Design review of the part built by this model. Coordinates are the model's own, in mm. A direction names the side the tool comes from. Coordinates: 2 decimals unless noted, no trailing zeros. Write each loop counter-clockwise with the first axis right and the second up, starting at its lowest first coordinate (ties: lowest second). Pieces come first, ordered by that corner, then holes. Notation, with made-up numbers: (-14, 46.5) -> (13, 46.5) arc R32 ccw to (13, 72.5) -> close; hole circle Ø2 at (37, 37). An arc over 180 degrees is marked (long way). Answer in a Markdown table with one row per item. Add a question column.
Item 1: For faces 1 (the face through (47.03, 166.91, 82.79)), 2 (the face through (-1, 2, 0)), 3 (the face through (-1, 166.3, 45)), list the 3-axis set-ups (+Z, -Z, +X, -X, +Y, -Y) from which the entire face can be reached by the end or side of a thin tool; tool diameter is ignored.
Item 2: Take a section at B-B, the plane y = -145.5. Write out the cut boundary in (x, z), and give its area (3 significant figures).
Item 3: Draft analysis for pull direction X (two halves, no side actions). For faces 4 (the face through (-1, 167.5, 44)), 5 (the face through (-80, -2, 44)), 6 (the face through (-78.8, -2, 45)), state which applies: released by +X, released by -X, zero draft, split by the parting line, or undercut.
Item 4: Clearance check with flat-ended pins moving along their axes: P1, Ø1, axis at x = -79.5, y = 105.5, coming from the -Z side; P2, Ø4, axis at x = -18, y = -50, coming from the +Z side. State where each tip first meets the part, or that it passes through.
Item 5: To check wall thickness, follow line 1 (X direction, y = -45, z = 48.5); line 2 (Y direction, x = -41.5, z = 17.5); line 3 (X direction, y = 167, z = 85). State the ranges of each line that lie inside material, in increasing order.
Item 6: Take a section at A-A, the plane z = 42. Write out the cut boundary in (x, y), and give its area (3 significant figures).
from build123d import *

# Parameters (mm, degrees)
SKETCH1_W           = 160
SKETCH1_H           = 335
BOSS_EXTRUDE1_DEPTH = 90
SHELL1_T            = -1.2
SKETCH2_R           = 3
CUT_EXTRUDE1_DEPTH  = 10
CUT_EXTRUDE2_DEPTH  = 249.508048159


with BuildPart() as part:
    # Sketch1 → Boss-Extrude1 (new body)
    with BuildSketch(Plane.XY):
        Rectangle(SKETCH1_W, SKETCH1_H)
    extrude(amount=BOSS_EXTRUDE1_DEPTH)

    # Shell1
    shell1_openings = [part.faces().sort_by_distance(p)[0] for p in [
        (0, 0, 90),
    ]]
    offset(amount=SHELL1_T, openings=shell1_openings, kind=Kind.INTERSECTION)

    # Sketch2 → Cut-Extrude1 (cut)
    with BuildSketch(Plane(origin=(0, 167.5, 0), x_dir=(1, 0, 0), z_dir=(0, 1, 0))):
        with Locations(Location((-45, -85, 0), (0, 0, 270))):
            Circle(SKETCH2_R)
        with Locations(Location((-25, -85, 0), (0, 0, 270))):
            Circle(SKETCH2_R)
        with Locations(Location((25, -85, 0), (0, 0, 270))):
            Circle(SKETCH2_R)
        with Locations(Location((45, -85, 0), (0, 0, 270))):
            Circle(SKETCH2_R)
    extrude(amount=-CUT_EXTRUDE1_DEPTH, mode=Mode.SUBTRACT)

    # Sketch3 → Cut-Extrude2 (cut, through all)
    with BuildSketch(Plane.ZY.offset(80)):
        with BuildLine():
            Line((87.8, 106.5), (87.8, 103.5))
            ThreePointArc((87.8, 103.5), (85, 100.7), (82.2, 103.5))
            Line((82.2, 103.5), (82.2, 106.5))
            ThreePointArc((82.2, 106.5), (85, 109.3), (87.8, 106.5))
        make_face()
        with BuildLine():
            Line((87.8, -106.5), (87.8, -103.5))
            ThreePointArc((87.8, -103.5), (85, -100.7), (82.2, -103.5))
            Line((82.2, -103.5), (82.2, -106.5))
            ThreePointArc((82.2, -106.5), (85, -109.3), (87.8, -106.5))
        make_face()
    extrude(amount=-CUT_EXTRUDE2_DEPTH, mode=Mode.SUBTRACT)


solid = part.part
Answers:
| question | item | result |
|---|---|---|
| 1 | face 1 | +Y |
| 1 | face 2 | -Z, +X, -X, +Y, -Y |
| 1 | face 3 | +Z |
| 2 | outline | (-80, 0) -> (80, 0) -> (80, 90) -> (78.8, 90) -> (78.8, 1.2) -> (-78.8, 1.2) -> (-78.8, 90) -> (-80, 90) -> close |
| 2 | area | 405 mm^2 |
| 3 | face 4 | zero draft |
| 3 | face 5 | released by -X |
| 3 | face 6 | undercut |
| 4 | P1 | stops at z = 0 |
| 4 | P2 | stops at z = 1.2 |
| 5 | line 1 | x = -80 to -78.8, 78.8 to 80 |
| 5 | line 2 | y = -167.5 to -166.3, 166.3 to 167.5 |
| 5 | line 3 | x = -80 to -48, -42 to -28, -22 to 22, 28 to 42, 48 to 80 |
| 6 | outline | (-80, -167.5) -> (80, -167.5) -> (80, 167.5) -> (-80, 167.5) -> close; hole (-78.8, -166.3) -> (78.8, -166.3) -> (78.8, 166.3) -> (-78.8, 166.3) -> close |
| 6 | area | 1,180 mm^2 |
